```python
from build123d import *

# Parameters (mm, degrees)
SKETCH1_R               = 5
BOSS_EXTRUDE1_DEPTH     = 18
SKETCH2_R               = 6
BOSS_EXTRUDE2_DEPTH     = 2
BOSS_EXTRUDE3_START     = 17
SKETCH3_R               = 5
BOSS_EXTRUDE3_DEPTH     = 17
SKETCH4_W               = 1.979153599
SKETCH4_H               = 1
CUT_EXTRUDE1_DEPTH      = 10
CUT_EXTRUDE1_DEPTH_BACK = 10
SKETCH5_W               = 5.566789872
SKETCH5_H               = 10
CHAMFER1_SIZE           = 0.3


with BuildPart() as part:
    # Sketch1 → Boss-Extrude1 (new body)
    with BuildSketch(Plane.XY):
        Circle(SKETCH1_R)
    extrude(amount=BOSS_EXTRUDE1_DEPTH)

    # Sketch2 → Boss-Extrude2 (add)
    with BuildSketch(Plane(origin=(0, 0, 0), x_dir=(-1, 0, 0), z_dir=(0, 0, -1))):
        Circle(SKETCH2_R)
    extrude(amount=BOSS_EXTRUDE2_DEPTH)

    # Sketch3 → Boss-Extrude3 (add)
    with BuildSketch(Plane(origin=(0, 0, -2), x_dir=(-1, 0, 0), z_dir=(0, 0, -1)).offset(BOSS_EXTRUDE3_START)):
        Circle(SKETCH3_R)
    extrude(amount=-BOSS_EXTRUDE3_DEPTH)

    # Sketch4 → Cut-Revolve1 (revolve, cut)
    with BuildSketch(Plane(origin=(0, 0, 0), x_dir=(1, 0, 0), z_dir=(0, 1, 0))):
        with Locations((-5.6395768, 17.5)):
            Rectangle(SKETCH4_W, SKETCH4_H)
    revolve(axis=Axis((0, 0, -19), (0, 0, 1)), mode=Mode.SUBTRACT)

    # Sketch5 → Cut-Extrude1 (cut, two sides: drawn at the far end of the back side and taken through both)
    with BuildSketch(Plane(origin=(0, 0, 0), x_dir=(1, 0, 0), z_dir=(0, 1, 0)).offset(-CUT_EXTRUDE1_DEPTH_BACK)):
        with Locations((-7.283394936, -13)):
            Rectangle(SKETCH5_W, SKETCH5_H)
    extrude(amount=CUT_EXTRUDE1_DEPTH + CUT_EXTRUDE1_DEPTH_BACK, mode=Mode.SUBTRACT)

    # Chamfer1
    chamfer1_edges = [part.edges().sort_by_distance(p)[0] for p in [
        (5, 0, -19),
        (1.118033989, -4.873397172, 18),
        (6, 0, 0),
        (6, 0, -2),
    ]]
    chamfer(chamfer1_edges, length=CHAMFER1_SIZE)


solid = part.part
```
Can you work these out from the model? Positions are in its coordinate system, mm. A direction names the side the tool comes from. Round coordinates to 2 decimals unless told otherwise and drop trailing zeros. Loops run counter-clockwise (first coordinate to the right, second up) from the corner with the lowest first, then second, coordinate; pieces in that order, holes last.
Item 1: If we mould it in two halves opening along Z, with no side actions, what happens to faces 1 (the cylindrical face through (1.01, 4.54, -17.51)), 2 (the flat face through (0, 0, 18)), 3 (the cylindrical face through (1.08, -4.88, -18.35)), 4 (the flat face through (0, 0, -19))? For each: +Z half, -Z half, draft (parallel to the pull), parting line (faces both ways), or undercut.
Item 2: Which directions (+Z, -Z, +X, -X, +Y, -Y) give clear straight access to the entire face, cutting with the end or side of a thin tool? Please do faces 5 (the cylindrical face through (4.77, 1.5, 8.73)), 6 (the cylindrical face through (1.08, -4.88, -9.6)), 7 (the cylindrical face through (6, 0, -1)), 8 (the flat face through (-4.5, 0, 13)).
Item 3: Please list where these lines run through material, in increasing order: L1, parallel to Z at x = -1.5, y = -5.25; L2, parallel to X at y = -4.5, z = -3.5; L3, parallel to Z at x = 5.25, y = -2.5.
Item 4: Suppose I cut it at B-B, the plane x = 0. Write out the boundary of the cut face in (y, z), then the cut area to 3 significant figures.
Item 5: Suppose I cut it at C-C, the plane z = -5.5. Write out the boundary of the cut face in (x, y).
Item 6: Suppose I cut it at D-D, the plane z = 8.5. Write out the boundary of the cut face in (x, y).
Item 7: Will these pins go through, and if not, where does the flat tip stop? pin 1 Ø6 at (x, z) = (4.5, -1.5) entering from +Y; pin 2 Ø2 at (x, z) = (-4, -6.5) entering from -Y; pin 3 Ø2 at (y, z) = (0.5, 14) entering from -X.
Reported:
1. face 1: undercut
1. face 2: +Z half
1. face 3: draft
1. face 4: -Z half
2. face 5: +Z
2. face 6: -Z
2. face 7: +Z, -Z
2. face 8: +Z, -X, +Y, -Y
3. L1: z = -2 to 0
3. L2: x = -2.18 to 2.18
3. L3: z = -1.89 to -0.11
4. outline: (-6, -1.7) - (-5.7, -2) - (-5, -2) - (-5, -17) - (-4.65, -17) - (-4.65, -18) - (-5, -18) - (-5, -18.7) - (-4.7, -19) - (4.7, -19) - (5, -18.7) - (5, -18) - (4.65, -18) - (4.65, -17) - (5, -17) - (5, -2) - (5.7, -2) - (6, -1.7) - (6, -0.3) - (5.7, 0) - (5, 0) - (5, 17.7) - (4.7, 18) - (-4.7, 18) - (-5, 17.7) - (-5, 0) - (-5.7, 0) - (-6, -0.3) - close
4. area: 373 mm2
5. outline: circle Ø10 at (0, 0)
6. outline: (-4.5, -2.18) arc R5 ccw (long way) to (-4.5, 2.18) - close
7. pin 1: stops at y = 5.81
7. pin 2: stops at y = -4
7. pin 3: stops at x = -4.5
